Input: dimensioned drawing with shaded views. Units: mm. Origin: part minimum x, y, z. A direction names the side the tool comes from. Give positions to 0.01 mm unless a question says otherwise; leave off trailing zeros. Order: outer loops, then holes, each group sorted by start corner. A loop starts at its lowest first (then second) coordinate and runs counter-clockwise, first axis right, second up. Notation, with made-up numbers: M -8.75,-22 L 36.25,-22 A23 cw 36.25,15 Z; hole C -36,54 d1. An arc over 180 degrees is marked long. Answer in a Markdown table with one row per item. Add a question column.
(1) Section query D-D, the plane z = 4.5. Return loops of the section in (x, y), plus the area to 3 significant figures.
(2) Section query C-C, the plane x = 25. Return loops of the section in (y, z), plus the area to 3 significant figures.
(3) Set-up query: the marked faces 1 and 2. Return all of +Z, -Z, +X, -X, +Y, -Y with unobstructed straight access to the full face (end or side cutting, diameter ignored); none if empty.
(4) Material intervals for line 1 along Z through (x, y) = (3, 6.75); line 2 along X through (y, z) = (7, 10.75); line 3 along Y through (x, z) = (17.5, 6), sorted ascending.
(5) Section query A-A, the plane z = 6.5. Return loops of the section in (x, y).
(6) Section query B-B, the plane y = 6.5. Return loops of the section in (x, z).
(7) Pin query (flat end, axial travel): P1, Ø2, axis at x = 26, y = 5.5, coming from the -Z side; P2, Ø1, axis at y = 10, z = 2, coming from the +X side; P3, Ø0.6, axis at y = 6.5, z = 4.5, coming from the -X side. Return the tip coordinate at first contact, or that it passes through.
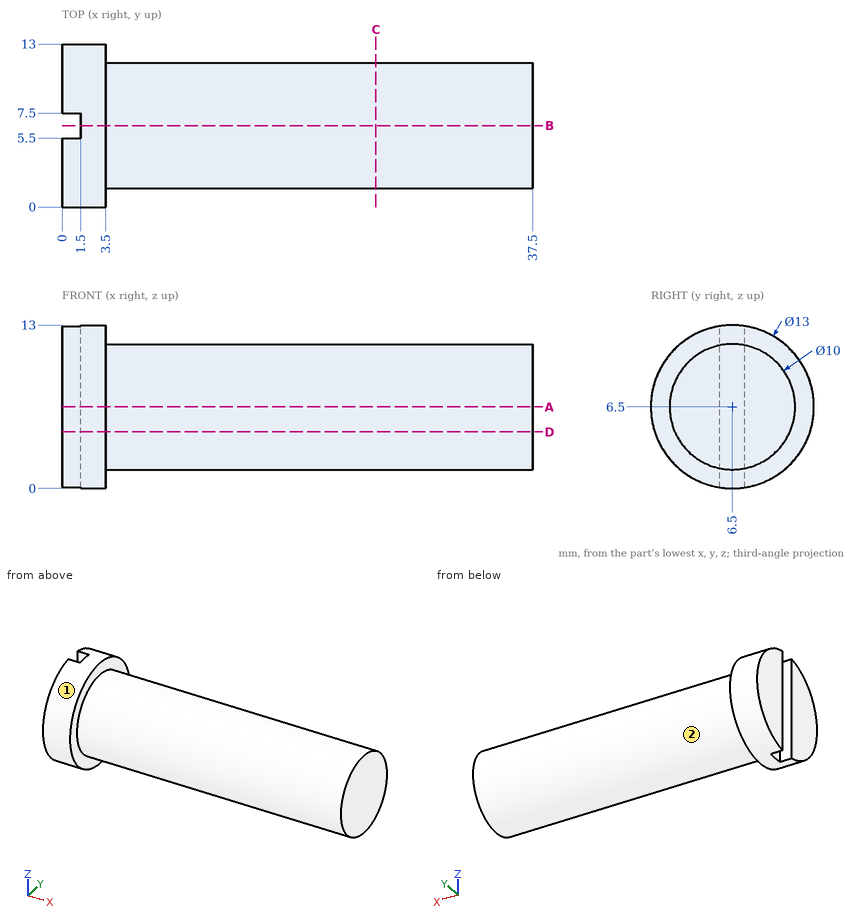
Values follow:
| question | item | result |
|---|---|---|
| 1 | outline | M 0,0.32 L 3.5,0.32 L 3.5,1.92 L 37.5,1.92 L 37.5,11.08 L 3.5,11.08 L 3.5,12.68 L 0,12.68 L 0,7.5 L 1.5,7.5 L 1.5,5.5 L 0,5.5 Z |
| 1 | area | 352 mm² |
| 2 | outline | C 6.5,6.5 d10 |
| 2 | area | 78.5 mm² |
| 3 | face 1 | +X, -X |
| 3 | face 2 | +X |
| 4 | line 1 | z = 0 to 13 |
| 4 | line 2 | x = 1.5 to 37.5 |
| 4 | line 3 | y = 1.53 to 11.47 |
| 5 | outline | M 0,0 L 3.5,0 L 3.5,1.5 L 37.5,1.5 L 37.5,11.5 L 3.5,11.5 L 3.5,13 L 0,13 L 0,7.5 L 1.5,7.5 L 1.5,5.5 L 0,5.5 Z |
| 6 | outline | M 1.5,0 L 3.5,0 L 3.5,1.5 L 37.5,1.5 L 37.5,11.5 L 3.5,11.5 L 3.5,13 L 1.5,13 Z |
| 7 | P1 | stops at z = 1.5 |
| 7 | P2 | stops at x = 3.5 |
| 7 | P3 | stops at x = 1.5 |
